from build123d import *

# Parameters (mm, degrees)
SKETCH1_W           = 101.6
SKETCH1_H           = 25.4
BOSS_EXTRUDE1_DEPTH = 1.524


with BuildPart() as part:
    # Sketch1 → Boss-Extrude1 (new body)
    with BuildSketch(Plane(origin=(0, 0, 0), x_dir=(1, 0, 0), z_dir=(0, 1, 0))):
        with Locations((50.8, 12.7)):
            Rectangle(SKETCH1_W, SKETCH1_H)
        with BuildLine():
            Line((11.049, 19.05), (19.018813647, 19.05))
            ThreePointArc((19.018813647, 19.05), (25.368813647, 12.7), (19.018813647, 6.35))
            Line((19.018813647, 6.35), (11.049, 6.35))
            ThreePointArc((11.049, 6.35), (4.699, 12.7), (11.049, 19.05))
        make_face(mode=Mode.SUBTRACT)
        with BuildLine():
            Line((80.899, 19.05), (88.868813647, 19.05))
            ThreePointArc((88.868813647, 19.05), (95.218813647, 12.7), (88.868813647, 6.35))
            Line((88.868813647, 6.35), (80.899, 6.35))
            ThreePointArc((80.899, 6.35), (74.549, 12.7), (80.899, 19.05))
        make_face(mode=Mode.SUBTRACT)
    extrude(amount=BOSS_EXTRUDE1_DEPTH)


solid = part.part
Geometry: final body of the model. Coordinates: model frame, mm. A direction names the side the tool comes from. Coordinates: 2 decimals unless noted, no trailing zeros. Loops run counter-clockwise (first coordinate to the right, second up) from the corner with the lowest first, then second, coordinate; pieces in that order, holes last. Notation, with made-up numbers: (8, -40) - (26, -40) arc R20 cw to (26, -18) - close; hole circle Ø10 at (-34, 86.5). An arc over 180 degrees is marked (long way). Put each result on its own line as item: value. Start each with the question number.
Q1. Cut plane C-C, the plane y = 0.85. Return loops of the section in (x, z), and give its area (3 significant figures).
Q2. Cut plane A-A, the plane z = -12.7. Return loops of the section in (x, y), and give its area (3 significant figures).
Q3. Set-up query: faces 1 (the flat face through (50, 1.524, -13)), 2 (the cylindrical face through (25.367, 0.751, -12.84)). Return all of +Z, -Z, +X, -X, +Y, -Y with unobstructed straight access to the full face (end or side cutting, diameter ignored); none if empty.
Q4. Line query: line 1 (X direction, y = 0.6, z = -13); line 2 (X direction, y = 0.8, z = -17.75); line 3 (Z direction, x = 13.5, y = 0.8). Output: solid intervals per line, ascending.
Q5. Cut plane B-B, the plane x = 18. Return loops of the section in (y, z).
Q6. Cut plane D-D, the plane x = 7.5. Return loops of the section in (y, z).
Q7. Pull-direction query (X, two-part tool) for faces 3 (the flat face through (50, 0, -13)), 4 (the cylindrical face through (95.217, 0.751, -12.84)); classes: released by +X, released by -X, zero draft, split by the parting line, or undercut.
Filled sheet:
1. outline: (0, -25.4) - (101.6, -25.4) - (101.6, 0) - (0, 0) - close; hole (11.05, -19.05) - (19.02, -19.05) arc R6.35 ccw to (19.02, -6.35) - (11.05, -6.35) arc R6.35 ccw to start; hole (80.9, -19.05) - (88.87, -19.05) arc R6.35 ccw to (88.87, -6.35) - (80.9, -6.35) arc R6.35 ccw to start
1. area: 2,120 mm²
2. outline: (0, 0) - (4.7, 0) - (4.7, 1.52) - (0, 1.52) - close; (25.37, 0) - (74.55, 0) - (74.55, 1.52) - (25.37, 1.52) - close; (95.22, 0) - (101.6, 0) - (101.6, 1.52) - (95.22, 1.52) - close
2. area: 91.8 mm²
3. face 1: +Z, -Z, +X, -X, +Y
3. face 2: +Y, -Y
4. line 1: 0 to 4.71, 25.36 to 74.56, 95.21 to 101.6
4. line 2: 0 to 7.2, 22.87 to 77.05, 92.72 to 101.6
4. line 3: -25.4 to -19.05, -6.35 to 0
5. outline: (0, -25.4) - (1.52, -25.4) - (1.52, -19.05) - (0, -19.05) - close; (0, -6.35) - (1.52, -6.35) - (1.52, 0) - (0, 0) - close
6. outline: (0, -25.4) - (1.52, -25.4) - (1.52, -17.97) - (0, -17.97) - close; (0, -7.43) - (1.52, -7.43) - (1.52, 0) - (0, 0) - close
7. face 3: zero draft
7. face 4: undercut
